Input: part model. Units: mm. Frame: model coordinates. A direction names the side the tool comes from. Give positions to 0.01 mm unless a question says otherwise; leave off trailing zeros. Loops run counter-clockwise (first coordinate to the right, second up) from the corner with the lowest first, then second, coordinate; pieces in that order, holes last. Notation, with made-up numbers: M 50.5,-4.75 L 73.5,-4.75 A28 cw 73.5,21.25 Z; hole C 58.25,1 d11. An arc over 180 degrees is marked long. One line per item, written item: value. Start each with the question number.
(1) Pin query (flat end, axial travel): P1, Ø3, axis at x = -49, y = 30.5, coming from the -Z side; P2, Ø12, axis at y = 28.5, z = 9, coming from the -X side; P3, Ø2, axis at x = -10, z = -111.5, coming from the +Y side. Return the tip coordinate at first contact, or that it passes through.
(2) Section B-B on x = 52.5. Output: boundary loops of the cut face in (y, z).
(3) Ray query, line 1 along Y through (x, z) = (-52, -4); line 2 along Z through (x, y) = (18, 57.5); line 3 along Y through (x, z) = (-47, 154.5). Return the intervals inside material, ascending. Write a range as from..to.
(4) Access query for faces 1 (the flat face through (-1, 45, 7.5)), 2 (the flat face through (75, 40, 0)), 3 (the flat face through (-75, 40, 0)). Directions: +Z, -Z, +X, -X, +Y, -Y. A direction counts if a zero-diameter tool reaches every point of the face in a straight line with its end or side. Return the directions, or none.
(5) Section C-C on z = 69. Output: boundary loops of the cut face in (x, y).
(6) Section A-A on y = 50. Output: boundary loops of the cut face in (x, z).
(7) Section D-D on x = -102. Output: boundary loops of the cut face in (y, z), plus the area to 3 significant figures.
```python
from build123d import *

# Parameters (mm, degrees)
SKETCH1_W           = 250
SKETCH1_H           = 360
BOSS_EXTRUDE1_DEPTH = 20
SKETCH2_W           = 150
SKETCH2_H           = 15
BOSS_EXTRUDE2_DEPTH = 50
FILLET1_R           = 10
SKETCH3_R           = 10
CUT_EXTRUDE1_DEPTH  = 236.968747931


with BuildPart() as part:
    # Sketch1 → Boss-Extrude1 (new body)
    with BuildSketch(Plane(origin=(0, 0, 0), x_dir=(1, 0, 0), z_dir=(0, 1, 0))):
        Rectangle(SKETCH1_W, SKETCH1_H)
    extrude(amount=BOSS_EXTRUDE1_DEPTH)

    # Sketch2 → Boss-Extrude2 (add)
    with BuildSketch(Plane(origin=(0, 20, 0), x_dir=(1, 0, 0), z_dir=(0, 1, 0))):
        Rectangle(SKETCH2_W, SKETCH2_H)
    extrude(amount=BOSS_EXTRUDE2_DEPTH)

    # Fillet1
    fillet1_edges = [part.edges().sort_by_distance(p)[0] for p in [
        (-75, 70, 0),
        (75, 70, 0),
    ]]
    fillet(fillet1_edges, radius=FILLET1_R)

    # Sketch3 → Cut-Extrude1 (cut, through all)
    with BuildSketch(Plane.XY.offset(7.5)):
        with Locations((52.5, 50)):
            Circle(SKETCH3_R)
        with Locations((-52.5, 50)):
            Circle(SKETCH3_R)
    extrude(amount=-CUT_EXTRUDE1_DEPTH, mode=Mode.SUBTRACT)


solid = part.part
```
Output values:
1. P1: stops at z = -7.5
1. P2: stops at x = -75
1. P3: stops at y = 20
2. outline: M 0,-180 L 20,-180 L 20,-7.5 L 40,-7.5 L 40,7.5 L 20,7.5 L 20,180 L 0,180 Z; M 60,-7.5 L 70,-7.5 L 70,7.5 L 60,7.5 Z
3. line 1: y = 0..40.01, 59.99..70
3. line 2: z = -7.5..7.5
3. line 3: y = 0..20
4. face 1: +Z, +X, -X, +Y
4. face 2: +Z, -Z, +X, +Y
4. face 3: +Z, -Z, -X, +Y
5. outline: M -125,0 L 125,0 L 125,20 L -125,20 Z
6. outline: M -75,-7.5 L -62.5,-7.5 L -62.5,7.5 L -75,7.5 Z; M -42.5,-7.5 L 42.5,-7.5 L 42.5,7.5 L -42.5,7.5 Z; M 62.5,-7.5 L 75,-7.5 L 75,7.5 L 62.5,7.5 Z
7. outline: M 0,-180 L 20,-180 L 20,180 L 0,180 Z
7. area: 7,200 mm²
